The listing builds one solid part. Answer for the finished solid, in the listing's coordinates (mm). A direction names the side the tool comes from. Give positions to 0.01 mm unless a question says otherwise; leave off trailing zeros. Loops run counter-clockwise (first coordinate to the right, second up) from the corner with the lowest first, then second, coordinate; pieces in that order, holes last. Notation, with made-up numbers: M -10.5,69.5 L 32.5,69.5 A24 cw 32.5,89.5 Z; hole C 66.25,3.25 d8. An arc over 180 degrees is marked long. Return JSON: item names as keys, results as strings.
from build123d import *

# Parameters (mm, degrees)
EXTRUDE_371_DEPTH = 11.5
SKETCH_4_W        = 0.8
SKETCH_4_H        = 12.088457268
CHAMFER_2038_SIZE = 2
FILLET_2080_R     = 0.6


with BuildPart() as part:
    # 草图1 → Extrude 371 (new body)
    with BuildSketch(Plane(origin=(0, 0, 0), x_dir=(0, 0, -1), z_dir=(1, 0, 0))):
        Polygon((13.5, 7.794228634), (13.5, -7.794228634), (0, -15.588457268), (-13.5, -7.794228634), (-13.5, 7.794228634), (0, 15.588457268), align=None)
    extrude(amount=EXTRUDE_371_DEPTH)

    # 草图2 → 凸台-旋转1 (revolve)
    with BuildSketch(Plane.XY, mode=Mode.PRIVATE) as revolve_1_sk:
        Polygon((0, 0), (121.5, 0), (121.5, 6.835), (121.5, 9), (27.8072, 9), (0, 9), align=None)
    revolve(revolve_1_sk.sketch.rotate(Axis((0, 0, 0), (1, 0, 0)), 90), axis=Axis((0, 0, 0), (1, 0, 0)))

    # 草图3 → 切除-旋转1 (revolve, cut)
    with BuildSketch(Plane.XY):
        Polygon((0, 13.5), (4.092522712, 20.588457268), (4.092522712, 25.588457268), (-10, 25.588457268), (-10, 13.5), align=None)
    revolve(axis=Axis((0, 0, 0), (1, 0, 0)), mode=Mode.SUBTRACT)

    # 草图5 → 切除-旋转2 (revolve, cut)
    with BuildSketch(Plane.XY):
        Polygon((11.5, 13.5), (7.407477288, 20.588457268), (7.407477288, 25.588457268), (17.407477288, 25.588457268), (17.407477288, 13.5), align=None)
    revolve(axis=Axis((0, 0, 0), (1, 0, 0)), mode=Mode.SUBTRACT)

    # 草图4 → 切除-旋转3 (revolve, cut)
    with BuildSketch(Plane.XY, mode=Mode.PRIVATE) as cut_revolve_3_sk:
        with Locations((11.1, 19.544228634)):
            Rectangle(SKETCH_4_W, SKETCH_4_H)
    revolve(cut_revolve_3_sk.sketch.rotate(Axis((0, 0, 0), (1, 0, 0)), 270), axis=Axis((0, 0, 0), (1, 0, 0)), mode=Mode.SUBTRACT)

    # Chamfer 2038
    chamfer_2038_edges = [part.edges().sort_by_distance(p)[0] for p in [
        (121.5, 0, -9),
    ]]
    chamfer(chamfer_2038_edges, length=CHAMFER_2038_SIZE)

    # Fillet 2080
    fillet_2080_edges = [part.edges().sort_by_distance(p)[0] for p in [
        (11.5, 0, -9),
    ]]
    fillet(fillet_2080_edges, radius=FILLET_2080_R)


solid = part.part
(1) The part is cut by section A-A (x = 19). Determine the outline of the cut face in (y, z).
Values follow:
{"outline": "C 0,0 d18"}
(2) Straight lines are drawn through the part: line 1 along X through (y, z) = (11.5, 1.5); line 2 along Y through (x, z) = (8.5, -6.75); line 3 along Y through (x, z) = (93.5, -0.5). For each, find the intervals that lie inside material, in ascending order.
Values follow:
{"line 1": "0 to 11.5", "line 2": "-11.69 to 11.69", "line 3": "-8.99 to 8.99"}
(3) Given pin 1 (1.5 mm diameter, centred on x = 63, z = -3.5, fed in from -Y); pin 2 (6 mm diameter, centred on x = 45.5, z = 8.5, fed in from -Y); pin 3 (3.5 mm diameter, centred on y = 8, z = -10, fed in from +X); pin 4 (6 mm diameter, centred on y = 7.5, z = -3.5, fed in from +X), each flat-ended and moving along its own axis, determine where each tip first touches the part or whether it passes through.
Values follow:
{"pin 1": "y = -8.57", "pin 2": "y = -7.12", "pin 3": "x = 11.5", "pin 4": "x = 121.5"}
(4) A tool of negligible diameter and unlimited length cuts with its end or side. For faces 1 (the flat face through (10.7, 7, 12)), 2 (the flat face through (10.7, -7, 12)), 3 (the flat face through (10.7, 7, -12)), 4 (the flat face through (10.7, -7, -12)), 5 (the cylindrical face through (65.048, -6.083, -6.633)), from which of +Z, -Z, +X, -X, +Y, -Y can it reach the whole face along a straight path? Write none if from no direction.
Values follow:
{"face 1": "+Z, +X, +Y", "face 2": "+Z, +X, -Y", "face 3": "-Z, +X, +Y", "face 4": "-Z, +X, -Y", "face 5": "+X"}
